Geometry: final body of the model. Coordinates: model frame, mm. A direction names the side the tool comes from. Give positions to 0.01 mm unless a question says otherwise; leave off trailing zeros. Write each loop counter-clockwise with the first axis right and the second up, starting at its lowest first coordinate (ties: lowest second). Pieces come first, ordered by that corner, then holes. Notation, with made-up numbers: M 2.5,73 L 37.5,73 A10 cw 37.5,89 Z; hole C 30.25,71.5 d9. An arc over 180 degrees is marked long. Use a Markdown table: item, result. Add a question column.
1) Set-up query: faces 1 (the flat face through (-8, 2.614, -1)), 2 (the flat face through (11, 3, -3)). Return all of +Z, -Z, +X, -X, +Y, -Y with unobstructed straight access to the full face (end or side cutting, diameter ignored); none if empty.
2) Section C-C on y = -0.2. Return the cut outline in (x, z).
3) Section A-A on x = 0. Return the cut outline in (y, z).
4) Draft query along Z for faces 3 (the cylindrical face through (-3.604, 0.042, 11.446)), 4 (the flat face through (-8, -2.614, 1)), 5 (the flat face through (2, 3, -6)). Return one class per face: +Z half, -Z half, draft (parallel to the pull), parting line (faces both ways), or undercut.
5) Line query: line 1 (X direction, y = -0.45, z = 0); line 2 (Y direction, x = -9, z = -4.75); line 3 (X direction, y = 1.6, z = -4.25). Output: solid intervals per line, ascending.
6) Pin query (flat end, axial travel): pin 1 (2 mm diameter, centred on x = 2, y = -2, fed in from -Z); pin 2 (1 mm diameter, centred on x = -4.5, y = 0, fed in from +Z). Return the tip coordinate at first contact, or that it passes through.
7) Section B-B on z = 0. Return the cut outline in (x, y).
```python
from build123d import *


with BuildPart() as part:
    # 草图1 → 旋转1 (revolve)
    with BuildSketch(Plane.XY, mode=Mode.PRIVATE) as revolve_1_sk:
        Polygon((5.95, 3), (5.95, -3), (7.45, -3), (7.779393861, -2.61408735), (10.385769976, -2.61408735), (10.837899147, -3), (12, -3), (12, 3), (10.837899147, 3), (10.385769976, 2.61408735), (7.779393861, 2.61408735), (7.45, 3), align=None)
    revolve(revolve_1_sk.sketch.rotate(Axis((0, 19.601235698, 0), (0, -1, 0)), 90), axis=Axis((0, 19.601235698, 0), (0, -1, 0)))


solid = part.part
```
Found:
| question | item | result |
|---|---|---|
| 1 | face 1 | +Y |
| 1 | face 2 | +Z, -Z, +X, -X, +Y |
| 2 | outline | C 0,0 d24; hole C 0,0 d11.9 |
| 3 | outline | M -3,-12 L 3,-12 L 3,-10.84 L 2.61,-10.39 L 2.61,-7.78 L 3,-7.45 L 3,-5.95 L -3,-5.95 L -3,-7.45 L -2.61,-7.78 L -2.61,-10.39 L -3,-10.84 Z; M -3,5.95 L 3,5.95 L 3,7.45 L 2.61,7.78 L 2.61,10.39 L 3,10.84 L 3,12 L -3,12 L -3,10.84 L -2.61,10.39 L -2.61,7.78 L -3,7.45 Z |
| 4 | face 3 | parting line |
| 4 | face 4 | undercut |
| 4 | face 5 | draft |
| 5 | line 1 | -12 to -5.95, 5.95 to 12 |
| 5 | line 2 | -2.61 to 2.61 |
| 5 | line 3 | -11.22 to -4.16, 4.16 to 11.22 |
| 6 | pin 1 | z = -11.96 |
| 6 | pin 2 | z = 11.31 |
| 7 | outline | M -12,-3 L -10.84,-3 L -10.39,-2.61 L -7.78,-2.61 L -7.45,-3 L -5.95,-3 L -5.95,3 L -7.45,3 L -7.78,2.61 L -10.39,2.61 L -10.84,3 L -12,3 Z; M 5.95,-3 L 7.45,-3 L 7.78,-2.61 L 10.39,-2.61 L 10.84,-3 L 12,-3 L 12,3 L 10.84,3 L 10.39,2.61 L 7.78,2.61 L 7.45,3 L 5.95,3 Z |
